Can you work these out from the model? Positions are in its coordinate system, mm. A direction names the side the tool comes from. Coordinates: 2 decimals unless noted, no trailing zeros. Loops run counter-clockwise (first coordinate to the right, second up) from the corner with the lowest first, then second, coordinate; pieces in that order, holes last. Notation, with made-up numbers: M 0,4 L 23,4 A9 ccw 23,12 Z; hole C 49.5,-8.75 d3. An arc over 180 degrees is marked long. Answer as a JSON object with one key per item and string values. Group by question number.
Item 1: If I drill on line 1 (Y direction, x = -14.75, z = 381.5); line 2 (Z direction, x = -25.5, y = -30); line 3 (X direction, y = -42, z = 399.5), over which ranges is the centre line in solid material (lowest first)?
Item 2: Suppose I cut it at B-B (x = -8). Write out the boundary of the cut face in (y, z), then the cut area to 3 significant figures.
Item 3: I'm going to push a flat-ended pin straight in: pin 1 Ø19.5 at (y, z) = (-30, 35.5) entering from +X. Where does the tip first touch, or does it pass through?
Item 4: Suppose I cut it at C-C (z = 281.5). Write out the boundary of the cut face in (x, y).
Item 5: Which directions (+Z, -Z, +X, -X, +Y, -Y) give clear straight access to the entire face, cutting with the end or side of a thin tool? Please do faces 4 (the flat face through (-30, -30, 214)), 5 (the flat face through (-24, -30, 214)).
Item 6: We'd pull the mould along Z, two halves only. Please class faces 1 (the cylindrical face through (-27.04, -28.16, 27.2)), 2 (the flat face through (-26, -30, 0)), 3 (the flat face through (-15, 0, 214)): +Z half, -Z half, draft (parallel to the pull), parting line (faces both ways), or undercut.
Item 7: Suppose I cut it at A-A (y = -30). Write out the boundary of the cut face in (x, z).
```python
from build123d import *

# Parameters (mm, degrees)
BOSS_EXTRUDE1_DEPTH = 435
SKETCH2_R           = 8.5
CUT_EXTRUDE1_DEPTH  = 435
CUT_EXTRUDE2_DEPTH  = 435


with BuildPart() as part:
    # Sketch1 → Boss-Extrude1 (new body)
    with BuildSketch(Plane.XY):
        with BuildLine():
            Line((0, 0), (-30, 0))
            Line((-30, 0), (-30, -60))
            Line((-30, -60), (0, -60))
            Line((0, -60), (0, -58.715972734))
            ThreePointArc((0, -58.715972734), (-0.735871259, -56.747795647), (-2.582480697, -55.745168528))
            Line((-2.582480697, -55.745168528), (-18.835038606, -53.461020473))
            ThreePointArc((-18.835038606, -53.461020473), (-22.528257481, -51.455766235), (-24, -47.519412061))
            Line((-24, -47.519412061), (-24, -12.480587939))
            ThreePointArc((-24, -12.480587939), (-22.528257481, -8.544233765), (-18.835038606, -6.538979527))
            Line((-18.835038606, -6.538979527), (-2.582480697, -4.254831472))
            ThreePointArc((-2.582480697, -4.254831472), (-0.735871259, -3.252204353), (0, -1.284027266))
            Line((0, -1.284027266), (0, 0))
        make_face()
    extrude(amount=BOSS_EXTRUDE1_DEPTH)

    # Sketch2 → Cut-Extrude1 (cut)
    with BuildSketch(Plane.ZY.offset(30)):
        with Locations(Location((35.5, -30, 0), (0, 0, 270))):
            Circle(SKETCH2_R)
    extrude(amount=-CUT_EXTRUDE1_DEPTH, mode=Mode.SUBTRACT)

    # Sketch3 → Cut-Extrude2 (cut)
    with BuildSketch(Plane(origin=(0, 0, 0), x_dir=(1, 0, 0), z_dir=(0, 1, 0))):
        Polygon((-15, 0), (0, 0), (0, -35), align=None)
    extrude(amount=-CUT_EXTRUDE2_DEPTH, mode=Mode.SUBTRACT)


solid = part.part
```
From the geometry:
{
 "1": {"line 1": "-60 to -54.04, -5.96 to 0", "line 2": "0 to 27, 44 to 435", "line 3": "-30 to -24"},
 "2": {"outline": "M -60,16.33 L -54.98,16.33 L -54.98,435 L -60,435 Z; M -5.02,16.33 L 0,16.33 L 0,435 L -5.02,435 Z", "area": "4,200 mm2"},
 "3": {"pin 1": "x = -24"},
 "4": {"outline": "M -30,-60 L 0,-60 L 0,-58.72 A3 ccw -2.58,-55.75 L -18.84,-53.46 A6 cw -24,-47.52 L -24,-12.48 A6 cw -18.84,-6.54 L -2.58,-4.25 A3 ccw 0,-1.28 L 0,0 L -30,0 Z"},
 "5": {"face 4": "+Z, -Z, -X, +Y, -Y", "face 5": "+Z, -Z, +X"},
 "6": {"face 1": "undercut", "face 2": "-Z half", "face 3": "draft"},
 "7": {"outline": "M -30,0 L -24,0 L -24,27 L -30,27 Z; M -30,44 L -24,44 L -24,435 L -30,435 Z"}
}
